```python
from build123d import *

# Parameters (mm, degrees)
SKETCH1_R           = 1.6
BOSS_EXTRUDE1_DEPTH = 2
SKETCH2_R           = 1.6
SKETCH2_W           = 26.1
SKETCH2_H           = 9.6
CUT_EXTRUDE1_DEPTH  = 2
FILLET1_R           = 0.5


with BuildPart() as part:
    # Sketch1 → Boss-Extrude1 (new body)
    with BuildSketch(Plane(origin=(0, 0, 0), x_dir=(1, 0, 0), z_dir=(0, 1, 0))):
        with BuildLine():
            Line((-23.5, -13), (23.5, -13))
            ThreePointArc((23.5, -13), (24.914213562, -12.414213562), (25.5, -11))
            Line((25.5, -11), (25.5, 11))
            ThreePointArc((25.5, 11), (24.914213562, 12.414213562), (23.5, 13))
            Line((23.5, 13), (-23.5, 13))
            ThreePointArc((-23.5, 13), (-24.914213562, 12.414213562), (-25.5, 11))
            Line((-25.5, 11), (-25.5, -11))
            ThreePointArc((-25.5, -11), (-24.914213562, -12.414213562), (-23.5, -13))
        make_face()
        with Locations(Location((-22.5, 10, 0), (0, 0, 270))):
            Circle(SKETCH1_R, mode=Mode.SUBTRACT)
        with Locations(Location((22.5, 10, 0), (0, 0, 270))):
            Circle(SKETCH1_R, mode=Mode.SUBTRACT)
        with Locations(Location((22.5, -10, 0), (0, 0, 270))):
            Circle(SKETCH1_R, mode=Mode.SUBTRACT)
        with Locations(Location((-22.5, -10, 0), (0, 0, 270))):
            Circle(SKETCH1_R, mode=Mode.SUBTRACT)
    extrude(amount=BOSS_EXTRUDE1_DEPTH)

    # Sketch2 → Cut-Extrude1 (cut)
    with BuildSketch(Plane.XZ):
        with Locations(Location((-16.25, 0, 0), (0, 0, 270))):
            Circle(SKETCH2_R)
        with Locations(Location((17.311344744, 0, 0), (0, 0, 270))):
            Circle(SKETCH2_R)
        Rectangle(SKETCH2_W, SKETCH2_H)
    extrude(amount=-CUT_EXTRUDE1_DEPTH, mode=Mode.SUBTRACT)

    # Fillet1
    fillet1_edges = [part.edges().sort_by_distance(p)[0] for p in [
        (13.05, 1, 4.8),
        (13.05, 1, -4.8),
        (-13.05, 1, -4.8),
        (-13.05, 1, 4.8),
    ]]
    fillet(fillet1_edges, radius=FILLET1_R)


solid = part.part
```
The listing builds one solid part. Answer for the finished solid, in the listing's coordinates (mm). A direction names the side the tool comes from. Coordinates: 2 decimals unless noted, no trailing zeros. Loops run counter-clockwise (first coordinate to the right, second up) from the corner with the lowest first, then second, coordinate; pieces in that order, holes last. Notation, with made-up numbers: (68.25, 47.25) - (120.25, 47.25) arc R16 cw to (120.25, 56.25) - close; hole circle Ø9 at (37.5, 1.25). An arc over 180 degrees is marked (long way). Use a Markdown table: item, result. Add a question column.
1) The mould has two halves that part along X. Classify faces 3 (the flat face through (0, 1, 4.8)), 4 (the cylindrical face through (24.9, 0.99, 12.43)), 5 (the cylindrical face through (-24.93, 0.99, 12.4)): released by +X, released by -X, zero draft, split by the parting line, or undercut.
2) The part is cut by section C-C, the plane z = 0. Give the vertices of the cut face in (x, y), and give its area (3 significant figures).
3) Find the intervals of material crossed by line 1 (X direction, y = 0.6, z = -10); line 2 (X direction, y = 1.5, z = 0); line 3 (Z direction, x = 7, y = 0.75), in increasing order.
4) For faces 1 (the flat face through (-13.05, 1, 0)), 2 (the flat face through (0, 1, 13)), determine the directions among +Z, -Z, +X, -X, +Y, -Y from which every point of the face is accessible in a straight line to the end or side of a thin tool.
5) The part is cut by section D-D, the plane x = -22.5. Give the vertices of the cut face in (y, z).
6) The part is cut by section B-B, the plane z = 3.5. Give the vertices of the cut face in (x, y).
7) The part is cut by section A-A, the plane x = -16.25. Give the vertices of the cut face in (y, z).
Here are the results:
| question | item | result |
|---|---|---|
| 1 | face 3 | undercut |
| 1 | face 4 | released by +X |
| 1 | face 5 | released by -X |
| 2 | outline | (-25.5, 0) - (-17.85, 0) - (-17.85, 2) - (-25.5, 2) - close; (-14.65, 0) - (-13.05, 0) - (-13.05, 2) - (-14.65, 2) - close; (13.05, 0) - (15.71, 0) - (15.71, 2) - (13.05, 2) - close; (18.91, 0) - (25.5, 0) - (25.5, 2) - (18.91, 2) - close |
| 2 | area | 37.0 mm^2 |
| 3 | line 1 | x = -25.5 to -24.1, -20.9 to 20.9, 24.1 to 25.5 |
| 3 | line 2 | x = -25.5 to -17.85, -14.65 to -13.05, 13.05 to 15.71, 18.91 to 25.5 |
| 3 | line 3 | z = -13 to -4.8, 4.8 to 13 |
| 4 | face 1 | +Y, -Y |
| 4 | face 2 | +Z, +X, -X, +Y, -Y |
| 5 | outline | (0, -13) - (2, -13) - (2, -11.6) - (0, -11.6) - close; (0, -8.4) - (2, -8.4) - (2, 8.4) - (0, 8.4) - close; (0, 11.6) - (2, 11.6) - (2, 13) - (0, 13) - close |
| 6 | outline | (-25.5, 0) - (-13.05, 0) - (-13.05, 2) - (-25.5, 2) - close; (13.05, 0) - (25.5, 0) - (25.5, 2) - (13.05, 2) - close |
| 7 | outline | (0, -13) - (2, -13) - (2, -1.6) - (0, -1.6) - close; (0, 1.6) - (2, 1.6) - (2, 13) - (0, 13) - close |
